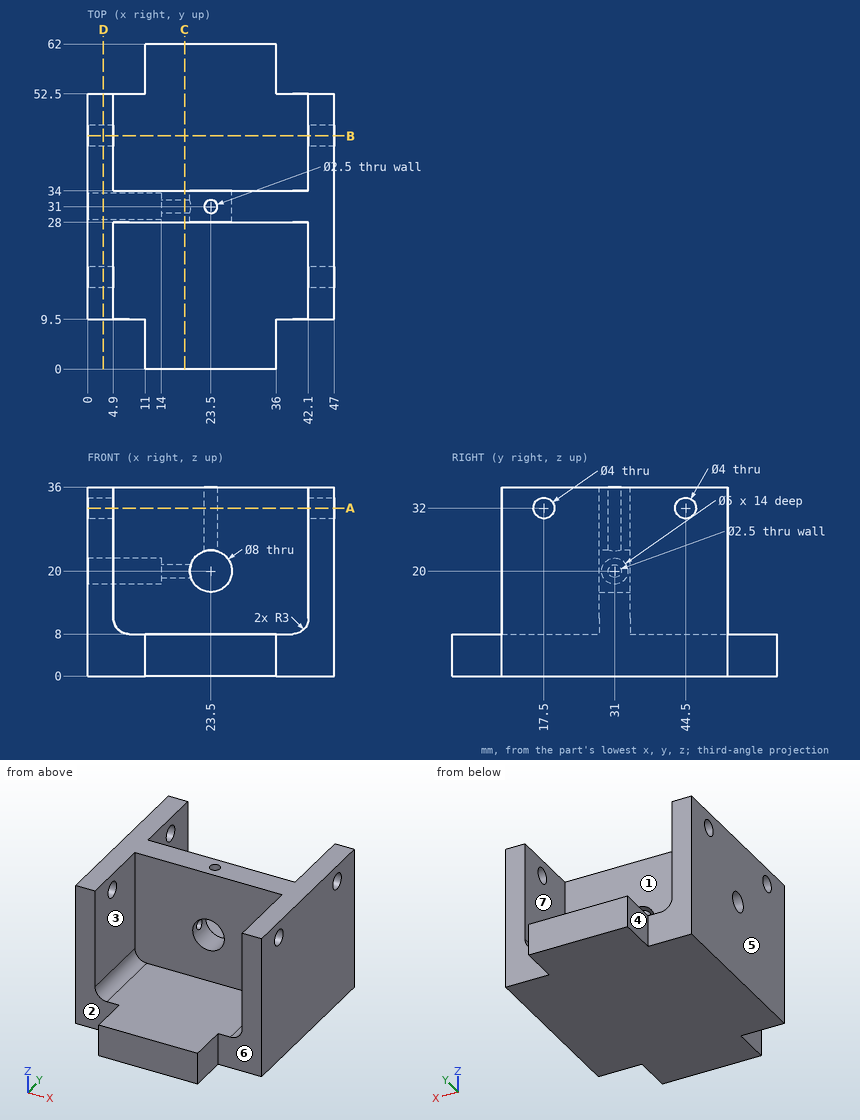
Design review of the part shown in the three views and the two pictorial views. Dimensions are in mm from the part's minimum x, y and z. A direction names the side the tool comes from. Give positions to 0.01 mm unless a question says otherwise; leave off trailing zeros. Order: outer loops, then holes, each group sorted by start corner. A loop starts at its lowest first (then second) coordinate and runs counter-clockwise, first axis right, second up. Notation, with made-up numbers: M 27.25,82.25 L 70.25,82.25 A16 ccw 70.25,87.25 Z; hole C 63.5,-25 d5. An arc over 180 degrees is marked long. Answer in a Markdown table with one row per item. Add a question column.
(1) For pin 1 (12 mm diameter, centred on x = 5, z = 20, fed in from -Y); pin 2 (5 mm diameter, centred on x = 23.5, z = 20, fed in from -Y); pin 3 (6.5 mm diameter, centred on y = 57, z = 5.5, fed in from +X); pin 4 (9 mm diameter, centred on x = 40.5, z = 18, fed in from +Y), all flat-tipped, find the tip position at first contact; note any pin that passes through.
(2) Consider section C-C on x = 18.5. State the section outline as (y, z) points.
(3) For the marked faces 1, 2, 3 and 4, list the 3-axis set-ups (+Z, -Z, +X, -X, +Y, -Y) from which the entire face can be reached by the end or side of a thin tool; tool diameter is ignored.
(4) Consider section D-D on x = 3. State the section outline as (y, z) points.
(5) Consider section A-A on z = 32. Give the number of separate pieces and of enclosed holes in the cut face, and give its area (3 significant figures).
(6) Consider section B-B on y = 44.5. State the section outline as (x, z) points.
(7) Mouldability with a two-part tool opening along X and no side actions: class the marked faces 5, 6 and 7 as +X half, -X half, draft (parallel to the pull), parting line (faces both ways), or undercut.
(8) Wall thickness on probe 1 along Y at (x, z) = (3.4, 32); probe 2 along X at (y, z) = (31, 29.75); probe 3 along X at (y, z) = (46.5, 31.5): over which ranges is each line inside the solid? List them lowest first. Write a range as [from, to].
Evaluation:
| question | item | result |
|---|---|---|
| 1 | pin 1 | stops at y = 9.5 |
| 1 | pin 2 | passes through |
| 1 | pin 3 | stops at x = 36 |
| 1 | pin 4 | stops at y = 52.5 |
| 2 | outline | M 0,0 L 62,0 L 62,8 L 34,8 L 34,36 L 28,36 L 28,8 L 0,8 Z; hole C 31,20 d2.5 |
| 3 | face 1 | +Z, +Y |
| 3 | face 2 | +Z, -Z, -X, -Y |
| 3 | face 3 | +Z, -Y |
| 3 | face 4 | +Z, -Z, -X, +Y |
| 4 | outline | M 9.5,0 L 52.5,0 L 52.5,36 L 9.5,36 Z; hole C 17.5,32 d4; hole C 31,20 d5; hole C 44.5,32 d4 |
| 5 | separate pieces | 5 |
| 5 | enclosed holes | 1 |
| 5 | area | 561 mm^2 |
| 6 | outline | M 0,0 L 47,0 L 47,30 L 42.1,30 L 42.1,11 A3 cw 39.1,8 L 7.9,8 A3 cw 4.9,11 L 4.9,30 L 0,30 Z; M 0,34 L 4.9,34 L 4.9,36 L 0,36 Z; M 42.1,34 L 47,34 L 47,36 L 42.1,36 Z |
| 7 | face 5 | -X half |
| 7 | face 6 | draft |
| 7 | face 7 | undercut |
| 8 | probe 1 | y = [9.5, 15.5], [19.5, 42.5], [46.5, 52.5] |
| 8 | probe 2 | x = [0, 22.25], [24.75, 47] |
| 8 | probe 3 | x = [0, 4.9], [42.1, 47] |
